The listing builds one solid part. Answer for the finished solid, in the listing's coordinates (mm). A direction names the side the tool comes from. Round coordinates to 2 decimals unless told otherwise and drop trailing zeros. Loops run counter-clockwise (first coordinate to the right, second up) from the corner with the lowest first, then second, coordinate; pieces in that order, holes last. Notation, with made-up numbers: M 13.25,-10 L 21.25,-10 A15 ccw 21.25,-1 Z; hole C 57,75 d9. An arc over 180 degrees is marked long. Answer as a JSON object with one key per item and string values.
```python
from build123d import *

# Parameters (mm, degrees)
SKETCH1_R           = 3.175
SKETCH1_W           = 63.5
SKETCH1_H           = 3.175
BOSS_EXTRUDE1_DEPTH = 3.175
SKETCH2_W           = 63.5
SKETCH2_H           = 3.175
BOSS_EXTRUDE2_DEPTH = 25.4
CUT_EXTRUDE1_DEPTH  = 106.992419611
SKETCH4_R           = 3.175
CUT_EXTRUDE2_DEPTH  = 25.4


with BuildPart() as part:
    # Sketch1 → Boss-Extrude1 (new body)
    # profile 1 of 2: a face of its own
    with BuildSketch(Plane(origin=(0, 0, 0), x_dir=(0, 0, -1), z_dir=(1, 0, 0))):
        with BuildLine():
            Line((0, 77.51210968), (0, 3.175))
            Line((0, 3.175), (63.5, 3.175))
            Line((63.5, 3.175), (63.5, 15.875))
            Line((63.5, 15.875), (15.080341671, 64.294658329))
            ThreePointArc((15.080341671, 64.294658329), (8.505408108, 64.65221549), (11.339511683, 70.595737627))
            ThreePointArc((11.339511683, 70.595737627), (12.906539417, 71.462906002), (13.511840983, 73.148482141))
            ThreePointArc((13.511840983, 73.148482141), (9.242521041, 80.072259125), (1.120938967, 79.618733943))
            ThreePointArc((1.120938967, 79.618733943), (0.297678098, 78.705253631), (0, 77.51210968))
        make_face()
        with Locations((9.525, 22.225)):
            Circle(SKETCH1_R, mode=Mode.SUBTRACT)
        with Locations((41.275, 22.225)):
            Circle(SKETCH1_R, mode=Mode.SUBTRACT)
        with Locations((9.525, 53.975)):
            Circle(SKETCH1_R, mode=Mode.SUBTRACT)
    # profile 2 of 2: a face of its own
    with BuildSketch(Plane(origin=(0, 0, 0), x_dir=(0, 0, -1), z_dir=(1, 0, 0))):
        with Locations((31.75, 1.5875)):
            Rectangle(SKETCH1_W, SKETCH1_H)
    extrude(amount=-BOSS_EXTRUDE1_DEPTH)

    # Sketch2 → Boss-Extrude2 (add)
    with BuildSketch(Plane(origin=(0, 0, 0), x_dir=(0, 0, -1), z_dir=(1, 0, 0))):
        with Locations((31.75, 1.5875)):
            Rectangle(SKETCH2_W, SKETCH2_H)
    extrude(amount=BOSS_EXTRUDE2_DEPTH)

    # Sketch3 → Cut-Extrude1 (cut, through all)
    with BuildSketch(Plane.XY):
        with BuildLine():
            ThreePointArc((-0.635, 0), (-2.431051224, 0.743948776), (-3.175, 2.54))
            Line((-3.175, 2.54), (-3.175, 0))
            Line((-3.175, 0), (-0.635, 0))
        make_face()
    extrude(amount=-CUT_EXTRUDE1_DEPTH, mode=Mode.SUBTRACT)

    # Sketch4 → Cut-Extrude2 (cut)
    with BuildSketch(Plane(origin=(0, 3.175, 0), x_dir=(1, 0, 0), z_dir=(0, 1, 0))):
        with Locations(Location((15.875, 53.975, 0), (0, 0, 270))):
            Circle(SKETCH4_R)
        with Locations(Location((12.7, 31.75, 0), (0, 0, 270))):
            Circle(SKETCH4_R)
        with Locations(Location((15.875, 9.525, 0), (0, 0, 270))):
            Circle(SKETCH4_R)
    extrude(amount=-CUT_EXTRUDE2_DEPTH, mode=Mode.SUBTRACT)


solid = part.part
```
Item 1: Straight lines are drawn through the part: line 1 (Y direction, x = 17, z = -27) (3 decimals); line 2 (X direction, y = 27, z = -50) (3 decimals). For each, find the intervals that lie inside material, in ascending order.
Values follow:
{"line 1": "0 to 3.175", "line 2": "-3.175 to 0"}
Item 2: The part is cut by section D-D (z = -40). Give the vertices of the cut face in (x, y) (3 decimals).
Values follow:
{"outline": "M -3.175,2.54 A2.54 ccw -0.635,0 L 25.4,0 L 25.4,3.175 L 0,3.175 L 0,19.317 L -3.175,19.317 Z; M -3.175,25.133 L 0,25.133 L 0,39.375 L -3.175,39.375 Z"}
Item 3: Which of the six approach directions +Z, -Z, +X, -X, +Y, -Y give full straight-line access (tool end or side, diameter ignored) to faces 1 (the face through (7, 3.175, -31)), 2 (the face through (-1.565, 80.016, -9.348))?
Values follow:
{"face 1": "+Z, -Z, +X, +Y", "face 2": "+X, -X, +Y"}
Item 4: The part is cut by section B-B (z = -26). Give the vertices of the cut face in (x, y) (3 decimals), then the cut area to 3 significant figures.
Values follow:
{"outline": "M -3.175,2.54 A2.54 ccw -0.635,0 L 25.4,0 L 25.4,3.175 L 0,3.175 L 0,53.375 L -3.175,53.375 Z", "area": "249 mm^2"}
Item 5: The part is cut by section C-C (x = 1). Give the vertices of the cut face in (y, z) (3 decimals).
Values follow:
{"outline": "M 0,-63.5 L 3.175,-63.5 L 3.175,0 L 0,0 Z"}
Item 6: Determine the mould class of faces 3 (the face through (-1.565, 78.721, -0.306)), 4 (the face through (16.015, 1.61, -12.697)), 5 (the face through (-3.175, 34, -24)) for opening direction X: released by +X, released by -X, zero draft, split by the parting line, or undercut.
Values follow:
{"face 3": "zero draft", "face 4": "undercut", "face 5": "released by -X"}
Item 7: The part is cut by section A-A (z = -53). Give the vertices of the cut face in (x, y) (3 decimals).
Values follow:
{"outline": "M -3.175,2.54 A2.54 ccw -0.635,0 L 12.853,0 L 12.853,3.175 L 0,3.175 L 0,26.375 L -3.175,26.375 Z; M 18.897,0 L 25.4,0 L 25.4,3.175 L 18.897,3.175 Z"}
Item 8: Flat-ended cylindrical pins translate along their axes: P1, Ø6, axis at x = 17.5, z = -34.5, coming from the +Y side (3 decimals); P2, Ø8, axis at y = 9, z = -49.5, coming from the +X side; P3, Ø5.5, axis at y = 22.225, z = -9.525, coming from the +X side. Find the tip coordinate at first contact, or state that the pin passes through.
Values follow:
{"P1": "y = 3.175", "P2": "x = 0", "P3": "through"}
